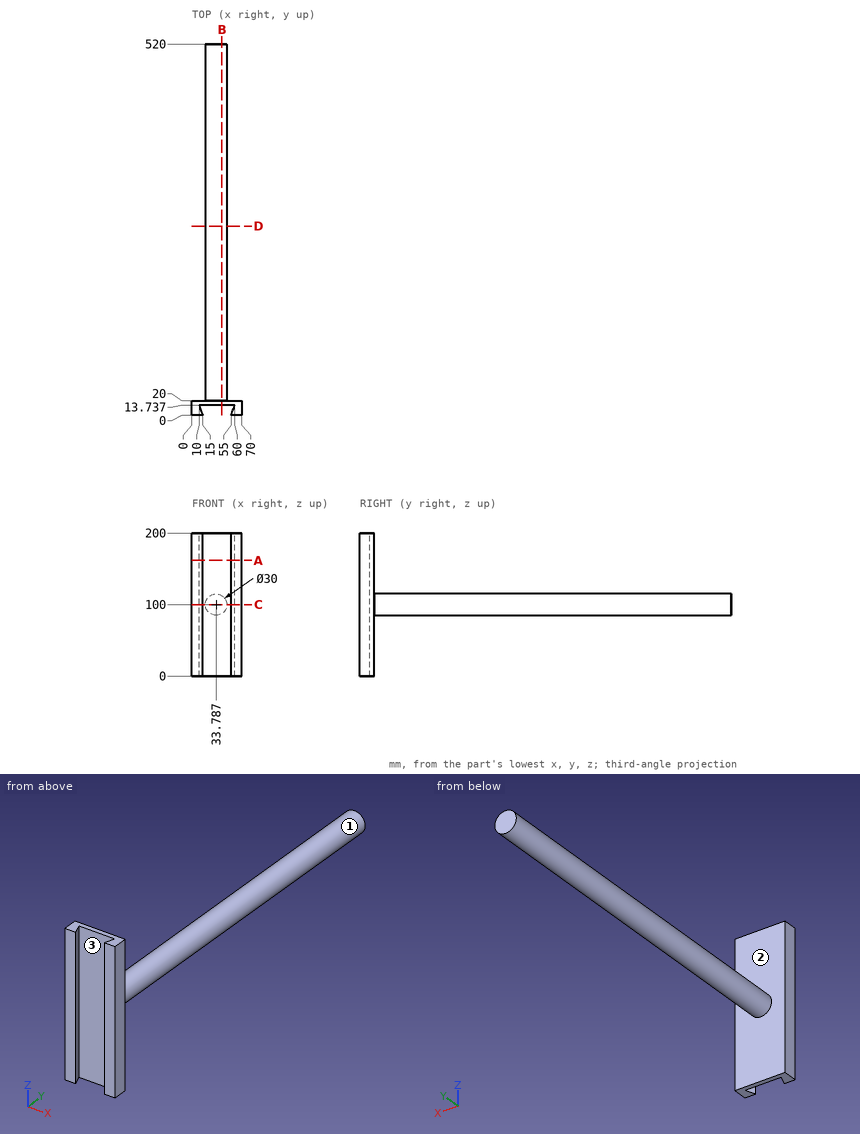
Print and shaded views of the part. All mm, measured from the part's lowest x, y and z. Give positions to 0.01 mm unless a question says otherwise; leave off trailing zeros. Loops run counter-clockwise (first coordinate to the right, second up) from the corner with the lowest first, then second, coordinate; pieces in that order, holes last. Notation, with made-up numbers: (50.25, 20) - (67.25, 20) arc R36 ccw to (67.25, 55) - close; hole circle Ø4 at (-9.5, -11.5). An arc over 180 degrees is marked (long way). Use a Markdown table: item, result.
(1) Band-saw the part on C-C (z = 100). Give the cut face in (x, y).
Taken from the geometry:
| item | result |
|---|---|
| outline | (0, 0) - (15, 0) - (10, 13.74) - (60, 13.74) - (55, 0) - (70, 0) - (70, 20) - (48.79, 20) - (48.79, 520) - (18.79, 520) - (18.79, 20) - (0, 20) - close |
(2) Band-saw the part on B-B (x = 42). Give the cut face in (y, z).
Taken from the geometry:
| item | result |
|---|---|
| outline | (13.74, 0) - (20, 0) - (20, 87.45) - (520, 87.45) - (520, 112.55) - (20, 112.55) - (20, 200) - (13.74, 200) - close |
(3) Pull direction X, two halves, no side cores. Call the marked faces 1, 2 and 3: +X half, -X half, draft (parallel to the pull), parting line (faces both ways), or undercut.
Taken from the geometry:
| item | result |
|---|---|
| face 1 | parting line |
| face 2 | draft |
| face 3 | undercut |
(4) Band-saw the part on A-A (z = 162). Give the cut face in (x, y).
Taken from the geometry:
| item | result |
|---|---|
| outline | (0, 0) - (15, 0) - (10, 13.74) - (60, 13.74) - (55, 0) - (70, 0) - (70, 20) - (0, 20) - close |
(5) Drop flat-ended pins along their axis: pin 1 Ø5 at (x, z) = (52.5, 177.5) entering from +Y; pin 2 Ø3 at (x, y) = (44.5, 218.5) entering from +Z; pin 3 Ø2 at (x, y) = (40, 366.5) entering from +Z (1 decimal). Give the stop position or say it passes through.
Taken from the geometry:
| item | result |
|---|---|
| pin 1 | y = 20 |
| pin 2 | z = 111.84 |
| pin 3 | z = 114.1 |
(6) Wall check: line 1 along Y through (x, z) = (21, 121); line 2 along Y through (x, z) = (25, 111); line 3 along Z through (x, y) = (34, 216.5). Give the ranges that are in metal, low to high.
Taken from the geometry:
| item | result |
|---|---|
| line 1 | 13.74 to 20 |
| line 2 | 13.74 to 520 |
| line 3 | 85 to 115 |
(7) Band-saw the part on D-D (y = 265). Give the cut face in (x, z).
Taken from the geometry:
| item | result |
|---|---|
| outline | circle Ø30 at (33.79, 100) |
